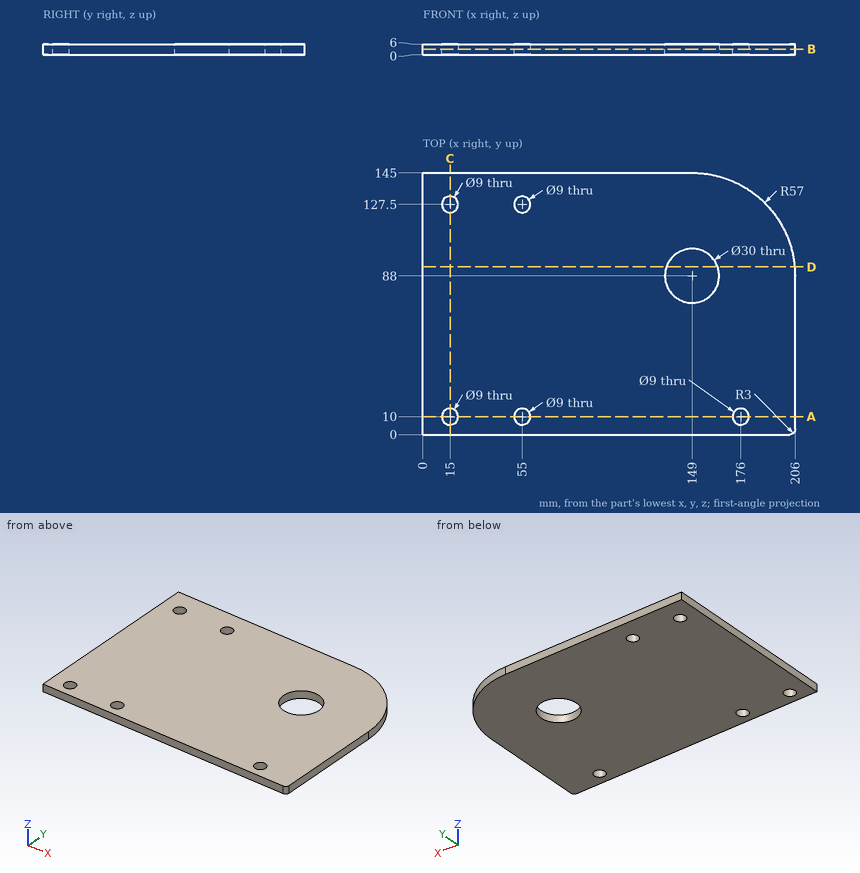
For this review, use the dimensioned drawing (mm, ordinates from the lowest corner) and the shaded views. Coordinates: 2 decimals unless noted, no trailing zeros. Loops run counter-clockwise (first coordinate to the right, second up) from the corner with the lowest first, then second, coordinate; pieces in that order, holes last. Notation, with made-up numbers: M 48.25,-29.5 L 107.25,-29.5 A13 cw 107.25,-10.5 Z; hole C -20.75,5 d8. An arc over 180 degrees is marked long. Answer as CSV lines item,"result".
Item 1: Add section C-C on x = 15. State the section outline as (y, z) points.
Answer list:
outline,"M 0,0 L 5.5,0 L 5.5,6 L 0,6 Z; M 14.5,0 L 123,0 L 123,6 L 14.5,6 Z; M 132,0 L 145,0 L 145,6 L 132,6 Z"
Item 2: Add section D-D on y = 93. State the section outline as (x, z) points.
Answer list:
outline,"M 0,0 L 134.86,0 L 134.86,6 L 0,6 Z; M 163.14,0 L 205.78,0 L 205.78,6 L 163.14,6 Z"
Item 3: For P1, Ø8, axis at x = 55, y = 127.5, coming from the +Z side, flat-tipped, find the tip position at first contact; note if it passes through.
Answer list:
P1,"through"
Item 4: For probe 1 along Y at (x, z) = (55, 1.3); probe 2 along Y at (x, z) = (53, 2.7); probe 3 along Y at (x, z) = (149.5, 2.65), list the stretches that pass through material, from the lowest coordinate up.
Answer list:
probe 1,"0 to 5.5, 14.5 to 123, 132 to 145"
probe 2,"0 to 5.97, 14.03 to 123.47, 131.53 to 145"
probe 3,"0 to 73.01, 102.99 to 145"
Item 5: Add section B-B on z = 3.1. State the section outline as (x, y) points.
Answer list:
outline,"M 0,0 L 203,0 A3 ccw 206,3 L 206,88 A57 ccw 149,145 L 0,145 Z; hole C 15,10 d9; hole C 15,127.5 d9; hole C 55,10 d9; hole C 55,127.5 d9; hole C 149,88 d30; hole C 176,10 d9"
Item 6: Add section A-A on y = 10. State the section outline as (x, z) points.
Answer list:
outline,"M 0,0 L 10.5,0 L 10.5,6 L 0,6 Z; M 19.5,0 L 50.5,0 L 50.5,6 L 19.5,6 Z; M 59.5,0 L 171.5,0 L 171.5,6 L 59.5,6 Z; M 180.5,0 L 206,0 L 206,6 L 180.5,6 Z"
